CAD build for the part. Positions are in the model's coordinates, mm. Round coordinates to 2 decimals unless told otherwise and drop trailing zeros. Loops run counter-clockwise (first coordinate to the right, second up) from the corner with the lowest first, then second, coordinate; pieces in that order, holes last. Notation, with made-up numbers: (29, 86) - (49, 86) arc R29 ccw to (49, 109) - close; hole circle Ø4 at (-36, 24). An arc over 180 degrees is marked (long way). One line per question, with ' | ' between items.
```python
from build123d import *

# Parameters (mm, degrees)
SKETCH1_W           = 300
SKETCH1_H           = 40
SKETCH1_R           = 12
BOSS_EXTRUDE1_DEPTH = 10
SKETCH2_W           = 22.25652502
SKETCH2_H           = 40
CUT_EXTRUDE1_DEPTH  = 10
FILLET1_R           = 10


with BuildPart() as part:
    # Sketch1 → Boss-Extrude1 (new body)
    with BuildSketch(Plane(origin=(0, 0, 0), x_dir=(1, 0, 0), z_dir=(0, 1, 0))):
        Rectangle(SKETCH1_W, SKETCH1_H)
        with Locations(Location((130, 0, 0), (0, 0, 270))):
            Circle(SKETCH1_R, mode=Mode.SUBTRACT)
        with Locations(Location((-5, 0, 0), (0, 0, 270))):
            Circle(SKETCH1_R, mode=Mode.SUBTRACT)
        with Locations(Location((-107, 0, 0), (0, 0, 270))):
            Circle(SKETCH1_R, mode=Mode.SUBTRACT)
    extrude(amount=BOSS_EXTRUDE1_DEPTH)

    # Sketch2 → Cut-Extrude1 (cut)
    with BuildSketch(Plane(origin=(0, 10, 0), x_dir=(1, 0, 0), z_dir=(0, 1, 0))):
        with Locations((-138.87173749, 0)):
            Rectangle(SKETCH2_W, SKETCH2_H)
    extrude(amount=-CUT_EXTRUDE1_DEPTH, mode=Mode.SUBTRACT)

    # Fillet1
    fillet1_edges = [part.edges().sort_by_distance(p)[0] for p in [
        (-127.74347498, 5, -20),
        (-127.74347498, 5, 20),
        (150, 5, 20),
        (150, 5, -20),
    ]]
    fillet(fillet1_edges, radius=FILLET1_R)


solid = part.part
```
(1) Cut at D-D, the plane z = 17. Write the cut outline in (x, y).
Results found:
outline: (-124.88, 0) - (147.14, 0) - (147.14, 10) - (-124.88, 10) - close
(2) Cut at A-A, the plane x = -107. Write the cut outline in (y, z).
Results found:
outline: (0, -20) - (10, -20) - (10, -12) - (0, -12) - close; (0, 12) - (10, 12) - (10, 20) - (0, 20) - close
(3) Cut at C-C, the plane z = 0. Write the cut outline in (x, y), then the cut area to 3 significant figures.
Results found:
outline: (-127.74, 0) - (-119, 0) - (-119, 10) - (-127.74, 10) - close; (-95, 0) - (-17, 0) - (-17, 10) - (-95, 10) - close; (7, 0) - (118, 0) - (118, 10) - (7, 10) - close; (142, 0) - (150, 0) - (150, 10) - (142, 10) - close | area: 2,060 mm²
(4) Two-plate mould, pull along Z, no slides. Class faces 1 (the face through (9, 10, 0)), 2 (the face through (-1.396, 4.93, 11.446)), 3 (the face through (146.99, 5.07, 17.15)), 4 (the face through (-103.396, 4.93, 11.446)): released by +Z, released by -Z, zero draft, split by the parting line, or undercut.
Results found:
face 1: zero draft | face 2: undercut | face 3: released by +Z | face 4: undercut
(5) Drop a flat-ended pin along its axis: P1, Ø21.5, axis at x = 130, z = 0, coming from the -Y side. Give the stop position or say it passes through.
Results found:
P1: passes through
(6) Probe L1, parallel to X at y = 6.25, z = 0; L2, parallel to X at y = 5.75, z = -9; L3, parallel to Z at x = -14.5, y = 3.25. List the from-to ranges inside material, lowest first.
Results found:
L1: x = -127.74 to -119, -95 to -17, 7 to 118, 142 to 150 | L2: x = -127.74 to -114.94, -99.06 to -12.94, 2.94 to 122.06, 137.94 to 150 | L3: z = -20 to -7.33, 7.33 to 20
(7) Cut at B-B, the plane y = 2.5. Write the cut outline in (x, z), then the cut area to 3 significant figures.
Results found:
outline: (-127.74, -10) arc R10 ccw to (-117.74, -20) - (140, -20) arc R10 ccw to (150, -10) - (150, 10) arc R10 ccw to (140, 20) - (-117.74, 20) arc R10 ccw to (-127.74, 10) - close; hole circle Ø24 at (-107, 0); hole circle Ø24 at (-5, 0); hole circle Ø24 at (130, 0) | area: 9,670 mm²
